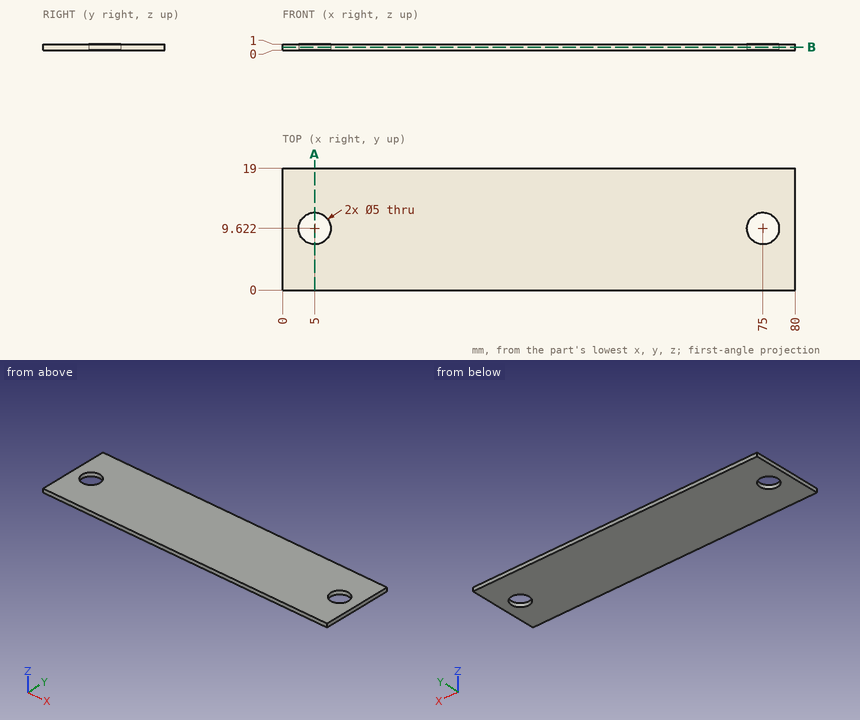
Input: dimensioned drawing with shaded views. Units: mm. Origin: part minimum x, y, z. Give positions to 0.01 mm unless a question says otherwise; leave off trailing zeros. Order: outer loops, then holes, each group sorted by start corner. A loop starts at its lowest first (then second) coordinate and runs counter-clockwise, first axis right, second up. Notation, with made-up numbers: (-11.75, -11.5) -> (13.25, -11.5) arc R13 ccw to (13.25, 0.5) -> close; hole circle Ø1 at (7.25, -24.5). An arc over 180 degrees is marked (long way). Use a Markdown table: item, result.
1) Section query B-B, the plane z = 0.5. Return the cut outline in (x, y).
Answer list:
| item | result |
|---|---|
| outline | (0, 0) -> (80, 0) -> (80, 19) -> (0, 19) -> close; hole circle Ø5 at (5, 9.62); hole circle Ø5 at (75, 9.62) |
2) Section query A-A, the plane x = 5. Return the cut outline in (y, z), then the cut area to 3 significant figures.
Answer list:
| item | result |
|---|---|
| outline | (0, 0) -> (7.12, 0) -> (7.12, 1) -> (0, 1) -> close; (12.12, 0) -> (19, 0) -> (19, 1) -> (12.12, 1) -> close |
| area | 14.0 mm² |
3) Ray query, line 1 along Y through (x, z) = (75, 0.8); line 2 along X through (y, z) = (10.75, 0.1); line 3 along X through (y, z) = (10.5, 0.6). Return the intervals inside material, ascending. Write a range as [from, to].
Answer list:
| item | result |
|---|---|
| line 1 | [0, 7.12], [12.12, 19] |
| line 2 | [0, 2.77], [7.23, 72.77], [77.23, 80] |
| line 3 | [0, 2.66], [7.34, 72.66], [77.34, 80] |
